CAD build for the part. Positions are in the model's coordinates, mm. Round coordinates to 2 decimals unless told otherwise and drop trailing zeros. Order: outer loops, then holes, each group sorted by start corner. A loop starts at its lowest first (then second) coordinate and runs counter-clockwise, first axis right, second up. Notation, with made-up numbers: (86.5, 52) -> (143.5, 52) arc R20 ccw to (143.5, 69) -> close; hole circle Ø3 at (-1, 13). An arc over 180 degrees is marked (long way). Return JSON: item names as keys, results as strings. Group by question number.
Q1. Flat gauge pin, fed straight in: pin 1 (3 mm diameter, centred on x = -92.5, z = 4, fed in from +Y). Where does the tip first touch, or does it go through?
Q2. Cut at A-A (z = 2.05). Write the cut outline in (x, y).
Q3. Probe line 1 along X through (y, z) = (-20, 3.45); line 2 along Y through (x, z) = (89, 2); line 3 along X through (y, z) = (-82, 4.75). List the from-to ranges inside material, lowest first.
Q4. Cut at B-B (x = -140). Write the cut outline in (y, z), then the cut area to 3 significant figures.
Q5. Cut at C-C (y = -11.5). Write the cut outline in (x, z), then the cut area to 3 significant figures.
from build123d import *

# Parameters (mm, degrees)
SKETCH1_W           = 400
SKETCH1_H           = 250
BOSS_EXTRUDE1_DEPTH = 5
SKETCH2_OUTSIDE_W   = 496.346
SKETCH2_OUTSIDE_H   = 346.346
CUT_EXTRUDE1_DEPTH  = 5


with BuildPart() as part:
    # Sketch1 → Boss-Extrude1 (new body)
    with BuildSketch(Plane.XY):
        Rectangle(SKETCH1_W, SKETCH1_H)
    extrude(amount=BOSS_EXTRUDE1_DEPTH)

    # Sketch2 outside → Cut-Extrude1 (cut)
    with BuildSketch(Plane.XY.offset(5)):
        Rectangle(SKETCH2_OUTSIDE_W, SKETCH2_OUTSIDE_H)
        Polygon((-200, -85), (-20, 125), (20, 125), (200, -85), (200, -125), (-200, -125), align=None, mode=Mode.SUBTRACT)
    extrude(amount=-CUT_EXTRUDE1_DEPTH, mode=Mode.SUBTRACT)


solid = part.part
Solution:
{
 "1": {"pin 1": "stops at y = 42.17"},
 "2": {"outline": "(-200, -125) -> (200, -125) -> (200, -85) -> (20, 125) -> (-20, 125) -> (-200, -85) -> close"},
 "3": {"line 1": "x = -144.29 to 144.29", "line 2": "y = -125 to 44.5", "line 3": "x = -197.43 to 197.43"},
 "4": {"outline": "(-125, 0) -> (-15, 0) -> (-15, 5) -> (-125, 5) -> close", "area": "550 mm²"},
 "5": {"outline": "(-137, 0) -> (137, 0) -> (137, 5) -> (-137, 5) -> close", "area": "1,370 mm²"}
}
